Read the model definition and answer for the solid it produces. Units are mm, in the model's axes. Face numbers are marked on the shaded views. A direction names the side the tool comes from. Give positions to 0.01 mm unless a question says otherwise; leave off trailing zeros. Order: outer loops, then holes, each group sorted by start corner. A loop starts at its lowest first (then second) coordinate and runs counter-clockwise, first axis right, second up. Notation, with made-up numbers: (9.5, -16) - (67.5, -16) arc R17 cw to (67.5, 7) - close; hole circle Ø8 at (77.5, -38). An arc over 180 degrees is marked (long way). Use a Markdown table: item, result. Add a question column.
1. Flat-ended cylindrical pins translate along their axes: P1, Ø1.5, axis at y = 0.5, z = 9, coming from the +X side; P2, Ø1.3, axis at x = 0.5, z = 10.5, coming from the +Y side; P3, Ø1, axis at y = -1, z = 8.5, coming from the -X side. Find the tip coordinate at first contact, or state that the pin passes through.
2. A cutting plane is placed at A-A on z = 7. Determine the outline of the cut face in (x, y), and give its area (3 significant figures).
3. A cutting plane is placed at B-B on z = 9. Determine the outline of the cut face in (x, y), and give its area (3 significant figures).
4. Consider L1, parallel to Z at x = 1.3, y = 0.5; L2, parallel to Y at x = -0.6, z = 3; L3, parallel to X at y = 0, z = 7. Determine where each line is inside the solid, lowest interval first.
5. Which of the six approach directions +Z, -Z, +X, -X, +Y, -Y give full straight-line access (tool end or side, diameter ignored) to the marked faces 1, 2 and 3?
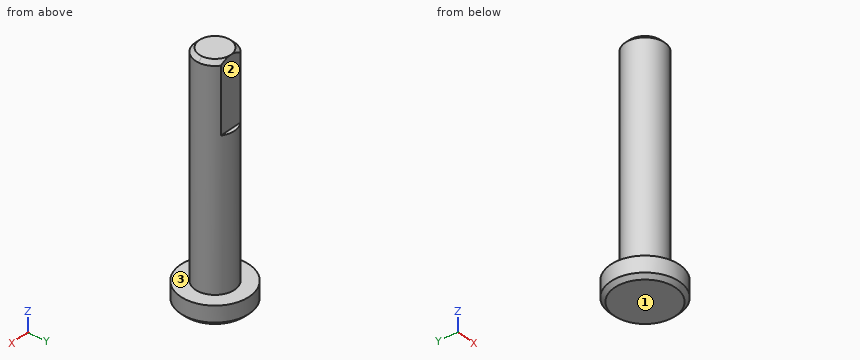
```python
from build123d import *

# Parameters (mm, degrees)
SKETCH1_R           = 1.75
BOSS_EXTRUDE1_DEPTH = 1
SKETCH2_R           = 1
BOSS_EXTRUDE2_DEPTH = 11
CHAMFER1_SIZE       = 0.2
CUT_EXTRUDE1_START  = -3.5
CUT_EXTRUDE1_DEPTH  = 3.5


with BuildPart() as part:
    # Sketch1 → Boss-Extrude1 (new body)
    with BuildSketch(Plane.XY):
        Circle(SKETCH1_R)
    extrude(amount=BOSS_EXTRUDE1_DEPTH)

    # Sketch2 → Boss-Extrude2 (add)
    with BuildSketch(Plane.XY.offset(1)):
        Circle(SKETCH2_R)
    extrude(amount=BOSS_EXTRUDE2_DEPTH)

    # Chamfer1
    chamfer1_edges = [part.edges().sort_by_distance(p)[0] for p in [
        (-1.75, 0, 0),
        (-1, 0, 12),
    ]]
    chamfer(chamfer1_edges, length=CHAMFER1_SIZE)

    # Sketch3 → Cut-Extrude1 (cut)
    with BuildSketch(Plane.XY.offset(12).offset(CUT_EXTRUDE1_START)):
        with BuildLine():
            Line((-0.6, 0.8), (0.6, 0.8))
            ThreePointArc((0.6, 0.8), (0, 1), (-0.6, 0.8))
        make_face()
    extrude(amount=CUT_EXTRUDE1_DEPTH, mode=Mode.SUBTRACT)


solid = part.part
```
Output values:
| question | item | result |
|---|---|---|
| 1 | P1 | x = 1 |
| 1 | P2 | y = 0.8 |
| 1 | P3 | x = -0.87 |
| 2 | outline | circle Ø2 at (0, 0) |
| 2 | area | 3.14 mm² |
| 3 | outline | (-0.6, 0.8) arc R1 ccw (long way) to (0.6, 0.8) - close |
| 3 | area | 2.98 mm² |
| 4 | L1 | 0 to 1 |
| 4 | L2 | -0.8 to 0.8 |
| 4 | L3 | -1 to 1 |
| 5 | face 1 | -Z, +X, -X, +Y, -Y |
| 5 | face 2 | +Z, +X, -X, +Y |
| 5 | face 3 | +Z |
